Input: part model. Units: mm. Frame: model coordinates. Face numbers are marked on the shaded views. Give positions to 0.01 mm unless a question says otherwise; leave off trailing zeros. Loops run counter-clockwise (first coordinate to the right, second up) from the corner with the lowest first, then second, coordinate; pieces in that order, holes last. Notation, with made-up numbers: M 70.25,30 L 111.25,30 A17 cw 111.25,35 Z; hole C 9.25,25 d9. An arc over 180 degrees is marked long. Return JSON: item names as keys, results as strings. Group by question number.
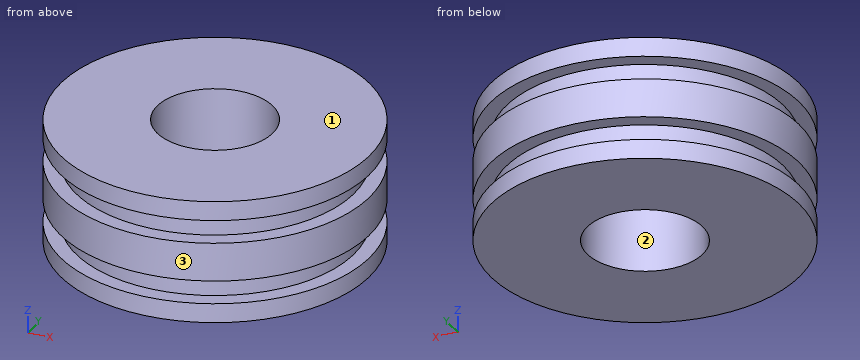
```python
from build123d import *

# Parameters (mm, degrees)
SKETCH_1_R          = 100
SKETCH_1_R_2        = 37.5
EXTRUDE_1_DEPTH     = 40
SKETCH_2_R          = 100
SKETCH_2_R_2        = 90
CUT_EXTRUDE_1_DEPTH = 7.5


with BuildPart() as part:
    # 草图1 → 凸台-拉伸1 (new, symmetric)
    with BuildSketch(Plane.XY):
        Circle(SKETCH_1_R)
        Circle(SKETCH_1_R_2, mode=Mode.SUBTRACT)
    extrude(amount=EXTRUDE_1_DEPTH, both=True)

    # 草图2 → 切除-拉伸1 (cut, symmetric)
    with BuildSketch(Plane.XY.offset(20)):
        Circle(SKETCH_2_R)
        Circle(SKETCH_2_R_2, mode=Mode.SUBTRACT)
    cut_extrude_1 = extrude(amount=CUT_EXTRUDE_1_DEPTH, both=True, mode=Mode.SUBTRACT)

    # 镜向1: 切除-拉伸1 across plane
    add(cut_extrude_1.mirror(Plane.XY), mode=Mode.SUBTRACT)


solid = part.part
```
Item 1: Material intervals for line 1 (Z direction, x = 37, y = 91); line 2 (Y direction, x = 0, z = 5); line 3 (Y direction, x = 0, z = -16.5), sorted ascending. Write a range as from..to.
Item 2: Pull-direction query (X, two-part tool) for the marked faces 1, 2 and 3; classes: pulls with the +X half, pulls with the -X half, needs draft (parallel to the pull), parting line crosses it, or undercut.
Item 3: Section C-C, the plane z = 23.5. Return loops of the section in (x, y), then the cut area to 3 significant figures.
Item 4: First-contact query: pin 1 Ø4 at (x, z) = (60, 18) entering from +Y; pin 2 Ø10 at (y, z) = (46.5, 15) entering from -X; pin 3 Ø1.5 at (y, z) = (38, -23) entering from +X. Flat tips, straight axial feed; report the tip coordinate or a pass-through.
Item 5: Section A-A, the plane x = 0. Return loops of the section in (y, z).
Item 6: Section D-D, the plane x = -77.5. Return loops of the section in (y, z).
Answer below:
{
 "1": {"line 1": "-40..-27.5, -12.5..12.5, 27.5..40", "line 2": "-100..-37.5, 37.5..100", "line 3": "-90..-37.5, 37.5..90"},
 "2": {"face 1": "needs draft", "face 2": "undercut", "face 3": "parting line crosses it"},
 "3": {"outline": "C 0,0 d180; hole C 0,0 d75", "area": "21,000 mm^2"},
 "4": {"pin 1": "y = 68.82", "pin 2": "x = -90.67", "pin 3": "x = 81.93"},
 "5": {"outline": "M -100,-40 L -37.5,-40 L -37.5,40 L -100,40 L -100,27.5 L -90,27.5 L -90,12.5 L -100,12.5 L -100,-12.5 L -90,-12.5 L -90,-27.5 L -100,-27.5 Z; M 37.5,-40 L 100,-40 L 100,-27.5 L 90,-27.5 L 90,-12.5 L 100,-12.5 L 100,12.5 L 90,12.5 L 90,27.5 L 100,27.5 L 100,40 L 37.5,40 Z"},
 "6": {"outline": "M -63.2,-40 L 63.2,-40 L 63.2,-27.5 L 45.76,-27.5 L 45.76,-12.5 L 63.2,-12.5 L 63.2,12.5 L 45.76,12.5 L 45.76,27.5 L 63.2,27.5 L 63.2,40 L -63.2,40 L -63.2,27.5 L -45.76,27.5 L -45.76,12.5 L -63.2,12.5 L -63.2,-12.5 L -45.76,-12.5 L -45.76,-27.5 L -63.2,-27.5 Z"}
}
